CAD build for the part. Positions are in the model's coordinates, mm. Face numbers are marked on the shaded views. A direction names the side the tool comes from. Give positions to 0.01 mm unless a question says otherwise; leave off trailing zeros. Loops run counter-clockwise (first coordinate to the right, second up) from the corner with the lowest first, then second, coordinate; pieces in that order, holes last.
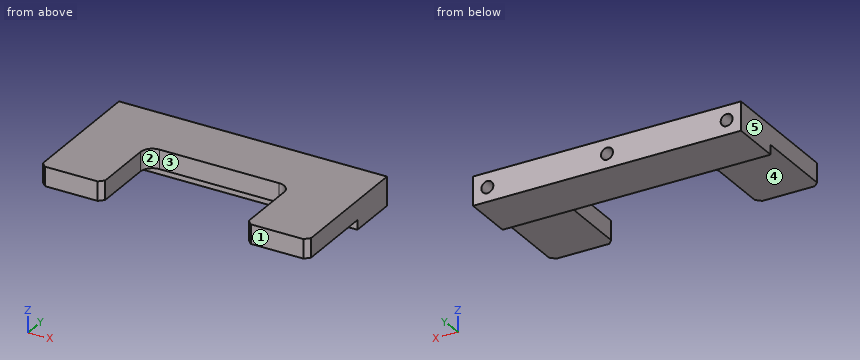
```python
from build123d import *

# Parameters (mm, degrees)
SKETCH1_W             = 112
SKETCH1_H             = 56
BOSS_EXTRUDE1_DEPTH   = 12
SKETCH2_W             = 112
SKETCH2_H             = 35
CUT_EXTRUDE1_DEPTH    = 4
M6_TAPPED_HOLE1_D     = 5
M6_TAPPED_HOLE1_DEPTH = 15
M6_TAPPED_HOLE1_TIP   = 1.502151548
SKETCH6_W             = 60
SKETCH6_H             = 32
CUT_EXTRUDE2_DEPTH    = 126.475097131
FILLET1_R             = 5
CHAMFER1_SIZE         = 2


with BuildPart() as part:
    # Sketch1 → Boss-Extrude1 (new body)
    with BuildSketch(Plane.XY):
        with Locations((56, 28)):
            Rectangle(SKETCH1_W, SKETCH1_H)
    extrude(amount=BOSS_EXTRUDE1_DEPTH)

    # Sketch2 → Cut-Extrude1 (cut)
    with BuildSketch(Plane(origin=(0, 0, 0), x_dir=(-1, 0, 0), z_dir=(0, 0, -1))):
        with Locations((-56, 17.5)):
            Rectangle(SKETCH2_W, SKETCH2_H)
    extrude(amount=-CUT_EXTRUDE1_DEPTH, mode=Mode.SUBTRACT)

    # M6 Tapped Hole1
    with Locations(Plane(origin=(0, 56, 0), x_dir=(1, 0, 0), z_dir=(0, 1, 0))):
        with Locations((106, -6), (6, -6), (56, -6)):
            Hole(M6_TAPPED_HOLE1_D / 2, depth=M6_TAPPED_HOLE1_DEPTH)
            with Locations((0, 0, -(M6_TAPPED_HOLE1_DEPTH + M6_TAPPED_HOLE1_TIP / 2))):  # 118° drill point
                Cone(0, M6_TAPPED_HOLE1_D / 2, M6_TAPPED_HOLE1_TIP, mode=Mode.SUBTRACT)

    # Sketch6 → Cut-Extrude2 (cut, through all)
    with BuildSketch(Plane(origin=(0, 0, 4), x_dir=(-1, 0, 0), z_dir=(0, 0, -1))):
        with Locations((-56, 16)):
            Rectangle(SKETCH6_W, SKETCH6_H)
    extrude(amount=-CUT_EXTRUDE2_DEPTH, mode=Mode.SUBTRACT)

    # Fillet1
    fillet1_edges = [part.edges().sort_by_distance(p)[0] for p in [
        (86, 32, 8),
        (26, 32, 8),
    ]]
    fillet(fillet1_edges, radius=FILLET1_R)

    # Chamfer1
    chamfer1_edges = [part.edges().sort_by_distance(p)[0] for p in [
        (86, 0, 8),
        (26, 0, 8),
        (112, 0, 8),
        (0, 0, 8),
    ]]
    chamfer(chamfer1_edges, length=CHAMFER1_SIZE)


solid = part.part
```
1. Saw through at A-A, the plane y = 46. List the corners of the cut face in (x, z).
Responses:
outline: (0, 0) - (112, 0) - (112, 12) - (0, 12) - close; hole circle Ø5 at (6, 6); hole circle Ø5 at (56, 6); hole circle Ø5 at (106, 6)
2. Probe line 1 along Z through (x, y) = (6, 47); line 2 along X through (y, z) = (23.5, 10.75); line 3 along X through (y, z) = (41.5, 7.75). List the from-to ranges inside material, lowest first.
Responses:
line 1: z = 0 to 3.5, 8.5 to 12
line 2: x = 0 to 26, 86 to 112
line 3: x = 0 to 4.21, 7.79 to 54.21, 57.79 to 104.21, 107.79 to 112
3. Drop flat-ended pins along their axis: pin 1 (2 mm diameter, centred on x = 20, y = 34.5, fed in from -Z); pin 2 (4.5 mm diameter, centred on x = 38, z = 1, fed in from -Y); pin 3 (4 mm diameter, centred on x = 106, z = 6, fed in from +Y); pin 4 (17.5 mm diameter, centred on x = 77.5, y = 25, fed in from -Z). Give the stop position or say it passes through.
Responses:
pin 1: stops at z = 0
pin 2: stops at y = 35
pin 3: stops at y = 40.7
pin 4: stops at z = 4
4. Tool access for the marked faces 1 and 2: list every direction of +Z, -Z, +X, -X, +Y, -Y with a clear straight run to the whole face (end or side of a thin tool).
Responses:
face 1: +Z, -Z, +X, -X, -Y
face 2: +Z, -Z, -Y
5. Pull direction X, two halves, no side cores. Call the marked faces 3, 4 and 5: released by +X, released by -X, zero draft, split by the parting line, or undercut.
Responses:
face 3: undercut
face 4: zero draft
face 5: released by -X
6. Saw through at C-C, the plane y = 7. List the corners of the cut face in (x, z), and give its area (3 significant figures).
Responses:
outline: (0, 4) - (26, 4) - (26, 12) - (0, 12) - close; (86, 4) - (112, 4) - (112, 12) - (86, 12) - close
area: 416 mm2
7. Saw through at D-D, the plane y = 29. List the corners of the cut face in (x, z).
Responses:
outline: (0, 4) - (26.42, 4) - (26.42, 12) - (0, 12) - close; (85.58, 4) - (112, 4) - (112, 12) - (85.58, 12) - close
8. Saw through at B-B, the plane x = 77.5. List the corners of the cut face in (y, z), and give its area (3 significant figures).
Responses:
outline: (32, 4) - (35, 4) - (35, 0) - (56, 0) - (56, 12) - (32, 12) - close
area: 276 mm2
